Could you check a few things on this model? Use its own coordinates, in mm. A direction names the side the tool comes from. Coordinates: 2 decimals unless noted, no trailing zeros. Loops run counter-clockwise (first coordinate to the right, second up) from the corner with the lowest first, then second, coordinate; pieces in that order, holes last.
from build123d import *

# Parameters (mm, degrees)
BOSS_EXTRUDE_DEPTH = 8.8
CHAMFER_2_SIZE     = 1.6


with BuildPart() as part:
    # Sketch1 → Boss-Extrude (new body)
    with BuildSketch(Plane(origin=(0, 0, 0), x_dir=(0, 0, -1), z_dir=(1, 0, 0))):
        Polygon((10.5, 6.062177826), (10.5, -6.062177826), (0, -12.124355653), (-10.5, -6.062177826), (-10.5, 6.062177826), (0, 12.124355653), align=None)
    extrude(amount=BOSS_EXTRUDE_DEPTH)

    # Sketch2 → Boss-Revolve1 (revolve)
    with BuildSketch(Plane.XY, mode=Mode.PRIVATE) as boss_revolve1_sk:
        Polygon((0, 0), (73.8, 0), (73.8, 5.268), (73.8, 7), (8.8, 7), (0, 7), align=None)
    revolve(boss_revolve1_sk.sketch.rotate(Axis((0, 0, 0), (-1, 0, 0)), 90), axis=Axis((0, 0, 0), (-1, 0, 0)))

    # Sketch3 → Cut-Revolve1 (revolve, cut)
    with BuildSketch(Plane.XY):
        Polygon((0, 10.5), (3.824573519, 17.124355653), (3.824573519, 22.124355653), (-10, 22.124355653), (-10, 10.5), align=None)
    revolve(axis=Axis((0, 0, 0), (1, 0, 0)), mode=Mode.SUBTRACT)

    # Sketch5 → Cut-Revolve2 (revolve, cut)
    with BuildSketch(Plane.XY):
        Polygon((8.8, 10.5), (4.975426481, 17.124355653), (4.975426481, 22.124355653), (14.975426481, 22.124355653), (14.975426481, 10.5), align=None)
    revolve(axis=Axis((0, 0, 0), (1, 0, 0)), mode=Mode.SUBTRACT)

    # Sketch4 → Cut-Revolve3 (revolve, cut)
    with BuildSketch(Plane.XY, mode=Mode.PRIVATE) as cut_revolve3_sk:
        Polygon((8.8, 9.517264973), (8.2, 9.863675135), (8.2, 22.124355653), (8.8, 22.124355653), align=None)
    revolve(cut_revolve3_sk.sketch.rotate(Axis((0, 0, 0), (1, 0, 0)), 90), axis=Axis((0, 0, 0), (1, 0, 0)), mode=Mode.SUBTRACT)

    # Chamfer 2
    chamfer_2_edges = [part.edges().sort_by_distance(p)[0] for p in [
        (73.8, 0, 7),
    ]]
    chamfer(chamfer_2_edges, length=CHAMFER_2_SIZE)

    # Sketch9 → Revolve1 (revolve)
    with BuildSketch(Plane.XY, mode=Mode.PRIVATE) as revolve1_sk:
        with BuildLine():
            Line((8.8, 7.6), (8.8, 7))
            Line((8.8, 7), (9.4, 7))
            ThreePointArc((9.4, 7), (8.975735931, 7.175735931), (8.8, 7.6))
        make_face()
    revolve(revolve1_sk.sketch.rotate(Axis((0, 0, 0), (1, 0, 0)), 90), axis=Axis((0, 0, 0), (1, 0, 0)))


solid = part.part
(1) Imagine slicing it at A-A, the plane x = 14. Write out the boundary of the cut face in (y, z).
Answers:
outline: circle Ø14 at (0, 0)
(2) Which directions (+Z, -Z, +X, -X, +Y, -Y) give clear straight access to the entire face, cutting with the end or side of a thin tool? Please do faces 1 (the face through (8.2, -9.5, 3.2)), 2 (the face through (73.8, 0, 0)).
Answers:
face 1: +X
face 2: +Z, -Z, +X, +Y, -Y
(3) For pin 1 (12 mm diameter, centred on x = 42.5, z = 6, fed in from -Y); pin 2 (12 mm diameter, centred on x = 18, y = 2, fed in from +Z); pin 3 (6 mm diameter, centred on y = 8.5, z = -1, fed in from +X), each with a flat end and sliding along its axis, tell me the tip position at first contact or that it passes through.
Answers:
pin 1: stops at y = -7
pin 2: stops at z = 7
pin 3: stops at x = 73.64
(4) I need wall thicknesses on probe 1 along X at (y, z) = (-5.25, 9); probe 2 along Z at (x, y) = (59, 0); probe 3 along Y at (x, z) = (26, -0.5). Which ranges of each line are inside material? Lowest first, please.
Answers:
probe 1: x = 0 to 8.2
probe 2: z = -7 to 7
probe 3: y = -6.98 to 6.98
